from build123d import *

# Parameters (mm, degrees)
BODY_PROFILE_SKETCH_R          = 25
BODY_PROFILE_SKETCH_R_2        = 9.5
BRACKET_BODY_EXTRUDE_110_DEPTH = 110
THROUGH_SLOT_CUT_DEPTH         = 110
ANGLED_BORE_SKETCH_46_R        = 23
ANGLED_BORE_46_DEPTH           = 55
MOUNTING_HOLES_SKETCH_R        = 5
MOUNTING_HOLES_4X_10_DEPTH     = 55


with BuildPart() as part:
    # Body Profile Sketch → Bracket Body Extrude 110 (new body)
    # profile 1 of 2: a face of its own
    with BuildSketch(Plane.XY):
        with BuildLine():
            Line((44, 0), (-44, 0))
            Line((-44, 0), (-44, -24))
            Line((-44, -24), (-19.769224603, -55.302867659))
            ThreePointArc((-19.769224603, -55.302867659), (-8.086080167, -16.343810376), (25, -40))
            ThreePointArc((25, -40), (23.656189624, -48.086080167), (19.769224603, -55.302867659))
            Line((19.769224603, -55.302867659), (44, -24))
            Line((44, -24), (44, 0))
        make_face()
    # profile 2 of 2: a face of its own
    with BuildSketch(Plane.XY):
        with Locations((0, -40)):
            Circle(BODY_PROFILE_SKETCH_R)
        with Locations((0, -40)):
            Circle(BODY_PROFILE_SKETCH_R_2, mode=Mode.SUBTRACT)
    extrude(amount=-BRACKET_BODY_EXTRUDE_110_DEPTH)

    # Through Slot Sketch → Through Slot Cut (cut)
    with BuildSketch(Plane(origin=(44, 0, 0), x_dir=(0, 0, -1), z_dir=(1, 0, 0))):
        with BuildLine():
            Line((12, -76.359959314), (12, -24))
            Line((12, -24), (75, -24))
            Line((75, -24), (75, -21))
            ThreePointArc((75, -21), (75.878679656, -18.878679656), (78, -18))
            Line((78, -18), (121.77138992, -18))
            Line((121.77138992, -18), (130.17802, -76.359959314))
            Line((130.17802, -76.359959314), (12, -76.359959314))
        make_face()
    extrude(amount=-THROUGH_SLOT_CUT_DEPTH, mode=Mode.SUBTRACT)

    # Angled Bore Sketch Ø46 → Angled Bore Ø46 (cut, symmetric)
    with BuildSketch(Plane(origin=(0, 0, 0), x_dir=(-1, 0, 0), z_dir=(0, 0.4226182617406939, -0.9063077870366526))):
        Circle(ANGLED_BORE_SKETCH_46_R)
    extrude(amount=ANGLED_BORE_46_DEPTH, both=True, mode=Mode.SUBTRACT)

    # Mounting Holes Sketch → Mounting Holes 4xØ10 (cut, symmetric)
    with BuildSketch(Plane(origin=(0, 0, 0), x_dir=(1, 0, 0), z_dir=(0, 1, 0))):
        with Locations(Location((-27.5, 95, 0), (0, 0, 180))):
            Circle(MOUNTING_HOLES_SKETCH_R)
        with Locations(Location((-27.5, 60, 0), (0, 0, 180))):
            Circle(MOUNTING_HOLES_SKETCH_R)
        with Locations(Location((27.5, 60, 0), (0, 0, 180))):
            Circle(MOUNTING_HOLES_SKETCH_R)
        with Locations(Location((27.5, 95, 0), (0, 0, 180))):
            Circle(MOUNTING_HOLES_SKETCH_R)
    extrude(amount=MOUNTING_HOLES_4X_10_DEPTH, both=True, mode=Mode.SUBTRACT)


solid = part.part
CAD build for the part. Positions are in the model's coordinates, mm. A direction names the side the tool comes from. Round coordinates to 2 decimals unless told otherwise and drop trailing zeros. Write each loop counter-clockwise with the first axis right and the second up, starting at its lowest first coordinate (ties: lowest second). Pieces come first, ordered by that corner, then holes.
(1) 3-axis set-ups, long thin cutter, end or side, ignore diameter. For faces 4 (the face through (-1, -9, -110)), 5 (the face through (1, -18, -94)): which of +Z, -Z, +X, -X, +Y, -Y reach the whole face in a straight line?
(2) Probe line 1 along Z through (x, y) = (27, -11); line 2 along Y through (x, z) = (-21.5, -95); line 3 along Z through (x, y) = (11, -45). List the from-to ranges inside material, lowest first.
(3) Slice it at D-D, the plane x = -27.5. Write the cut outline in (y, z), and give its area (3 significant figures).
(4) Slice it at A-A, the plane z = -60. Write the cut outline in (x, y), and give its area (3 significant figures).
(5) Slice it at C-C, the plane x = 1. Write the cut outline in (y, z), and give its area (3 significant figures).
(6) Mould opens along X. For faces 1 (the face through (0, -65, -6)), 2 (the face through (10, -40, -12)), 3 (the face through (-1.24, -30.58, -5.92)) say: pulls with the +X half, pulls with the -X half, needs draft (parallel to the pull), parting line crosses it, or undercut.
(7) Drop flat-ended pins along their axis: P1, Ø2.5, axis at x = 1, y = -22.5, coming from the -Z side; P2, Ø19, axis at x = 4, z = -56, coming from the -Y side; P3, Ø10, axis at x = -27, z = -93.5, coming from the -Y side. Give the stop position or say it passes through.
(8) Slice it at B-B, the plane y = -40. Write the cut outline in (x, z), and give its area (3 significant figures).
From the geometry:
1. face 4: -Z, +X, -X, +Y, -Y
1. face 5: -Z, +X, -X, -Y
2. line 1: z = -110 to -99.97, -90.03 to -64.97, -55.03 to 0
2. line 2: y = -18 to 0
2. line 3: z = -12 to 0
3. outline: (-45.32, -12) - (-24, -12) - (-24, -55) - (0, -55) - (0, 0) - (-45.32, 0) - close; (-24, -75) - (-21, -75) arc R3 cw to (-18, -78) - (-18, -90) - (0, -90) - (0, -65) - (-24, -65) - close; (-18, -110) - (0, -110) - (0, -100) - (-18, -100) - close
3. area: 2,270 mm2
4. outline: (-44, -24) - (-32.5, -24) - (-32.5, 0) - (-44, 0) - close; (-22.5, -24) - (22.5, -24) - (22.5, 0) - (-22.5, 0) - close; (32.5, -24) - (44, -24) - (44, 0) - (32.5, 0) - close
4. area: 1,630 mm2
5. outline: (-64.98, -12) - (-49.45, -12) - (-49.45, 0) - (-64.98, 0) - close; (-30.55, -12) - (-24, -12) - (-24, -75) - (-21, -75) arc R3 cw to (-18, -78) - (-18, -110) - (0, -110) - (0, -54.37) - (-25.35, 0) - (-30.55, 0) - close
5. area: 2,010 mm2
6. face 1: parting line crosses it
6. face 2: needs draft
6. face 3: undercut
7. P1: stops at z = -75
7. P2: stops at y = -24
7. P3: stops at y = -18
8. outline: (-31.61, -12) - (-9.5, -12) - (-9.5, 0) - (-31.61, 0) - close; (9.5, -12) - (31.61, -12) - (31.61, 0) - (9.5, 0) - close
8. area: 531 mm2
